from build123d import *

# Parameters (mm, degrees)
SKETCH1_R           = 8
BOSS_EXTRUDE1_DEPTH = 35
SKETCH2_W           = 18
SKETCH2_H           = 80
BOSS_EXTRUDE2_DEPTH = 24
FILLET1_R           = 5
SKETCH4_R           = 5
CUT_EXTRUDE1_DEPTH  = 57.115951386


with BuildPart() as part:
    # Sketch1 → Boss-Extrude1 (new body)
    with BuildSketch(Plane.XY):
        Circle(SKETCH1_R)
    extrude(amount=BOSS_EXTRUDE1_DEPTH)

    # Sketch2 → Boss-Extrude2 (add)
    with BuildSketch(Plane(origin=(0, 0, 0), x_dir=(-1, 0, 0), z_dir=(0, 0, -1))):
        Rectangle(SKETCH2_W, SKETCH2_H)
    extrude(amount=BOSS_EXTRUDE2_DEPTH)

    # Fillet1
    fillet1_edges = [part.edges().sort_by_distance(p)[0] for p in [
        (0, -40, 0),
        (0, 40, 0),
        (0, -40, -24),
        (0, 40, -24),
    ]]
    fillet(fillet1_edges, radius=FILLET1_R)

    # Sketch4 → Cut-Extrude1 (cut, through all)
    with BuildSketch(Plane.ZY.offset(9)):
        with Locations(Location((-12, -32, 0), (0, 0, 270))):
            Circle(SKETCH4_R)
        with Locations(Location((-12, 32, 0), (0, 0, 270))):
            Circle(SKETCH4_R)
    extrude(amount=-CUT_EXTRUDE1_DEPTH, mode=Mode.SUBTRACT)


solid = part.part
Could you check a few things on this model? Use its own coordinates, in mm. Coordinates: 2 decimals unless noted, no trailing zeros. Loops run counter-clockwise (first coordinate to the right, second up) from the corner with the lowest first, then second, coordinate; pieces in that order, holes last.
1. We'd pull the mould along Z, two halves only. Please class faces 1 (the face through (0, 37, -12)), 2 (the face through (-1.73, -7.81, 17.26)), 3 (the face through (0, 0, 35)): released by +Z, released by -Z, zero draft, split by the parting line, or undercut.
2. Imagine slicing it at A-A (y = -32). Please give me the cut outline in (x, z), and give its area (3 significant figures).
3. Imagine slicing it at C-C (x = 0). Please give me the cut outline in (y, z).
4. Imagine slicing it at D-D (y = -11). Please give me the cut outline in (x, z), and give its area (3 significant figures).
5. For P1, Ø3, axis at x = -0.5, z = 15.5, coming from the +Y side; P2, Ø2, axis at x = 1.5, z = 17.5, coming from the -Y side; P3, Ø1, axis at x = -1.5, z = 11, coming from the -Y side, each with a flat end and sliding along its axis, tell me the tip position at first contact or that it passes through.
6. Imagine slicing it at B-B (z = -8). Please give me the cut outline in (x, y).
7. I need wall thicknesses on L1, parallel to Z at x = 3.75, y = -32; L2, parallel to Z at x = 5.25, y = 8.5; L3, parallel to Z at x = 7.75, y = 28.5. Which ranges of each line are inside material? Lowest first, please.
Computed values:
1. face 1: undercut
1. face 2: zero draft
1. face 3: released by +Z
2. outline: (-9, -24) - (9, -24) - (9, -17) - (-9, -17) - close; (-9, -7) - (9, -7) - (9, 0) - (-9, 0) - close
2. area: 252 mm2
3. outline: (-40, -19) arc R5 ccw to (-35, -24) - (35, -24) arc R5 ccw to (40, -19) - (40, -5) arc R5 ccw to (35, 0) - (8, 0) - (8, 35) - (-8, 35) - (-8, 0) - (-35, 0) arc R5 ccw to (-40, -5) - close; hole circle Ø10 at (-32, -12); hole circle Ø10 at (32, -12)
4. outline: (-9, -24) - (9, -24) - (9, 0) - (-9, 0) - close
4. area: 432 mm2
5. P1: stops at y = 8
5. P2: stops at y = -7.98
5. P3: stops at y = -7.94
6. outline: (-9, -40) - (9, -40) - (9, -35) - (-9, -35) - close; (-9, -29) - (9, -29) - (9, 29) - (-9, 29) - close; (-9, 35) - (9, 35) - (9, 40) - (-9, 40) - close
7. L1: z = -24 to -17, -7 to 0
7. L2: z = -24 to 0
7. L3: z = -24 to -15.57, -8.43 to 0
